from build123d import *


with BuildPart() as part:
    # Sketch1 → Revolve2 (revolve)
    with BuildSketch(Plane.XY, mode=Mode.PRIVATE) as revolve2_sk:
        with BuildLine():
            Line((-2, 0), (-2, 53.291796068))
            ThreePointArc((-2, 53.291796068), (-5.61248608, 55.816699867), (-7, 60))
            Line((-7, 60), (-8, 60))
            Line((-8, 60), (-8, 8.392398037))
            Line((-8, 8.392398037), (-6.75, 8.392398037))
            ThreePointArc((-6.75, 8.392398037), (-6.244894811, 3.375866985), (-2.5, 0))
            Line((-2.5, 0), (-2, 0))
        make_face()
    revolve(revolve2_sk.sketch.rotate(Axis((0, 0, 0), (0, 1, 0)), 270), axis=Axis((0, 0, 0), (0, 1, 0)))


solid = part.part
Could you check a few things on this model? Use its own coordinates, in mm. A direction names the side the tool comes from. Give positions to 0.01 mm unless a question says otherwise; leave off trailing zeros. Loops run counter-clockwise (first coordinate to the right, second up) from the corner with the lowest first, then second, coordinate; pieces in that order, holes last. Notation, with made-up numbers: (50, 11) -> (96, 11) arc R20 ccw to (96, 23) -> close; hole circle Ø7 at (-14, 78.5). An arc over 180 degrees is marked (long way). Return JSON: item names as keys, results as strings.
Item 1: If we section it at D-D on z = -5: List the corners of the cut face in (x, y) for me (3 decimals), plus the area to 3 significant figures.
Geometry results:
{"outline": "(-6.245, 8.392) -> (-4.535, 8.392) arc R4.899 ccw (long way) to (4.535, 8.392) -> (6.245, 8.392) -> (6.245, 60) -> (4.899, 60) arc R4.899 cw to (-4.899, 60) -> (-6.245, 60) -> close", "area": "662 mm²"}
Item 2: If we section it at C-C on y = 19: List the corners of the cut face in (x, z) for me, plus the area to 3 significant figures.
Geometry results:
{"outline": "circle Ø16 at (0, 0); hole circle Ø4 at (0, 0)", "area": "188 mm²"}
Item 3: I'm going to push flat-ended pins straight in: pin 1 (4 mm diameter, centred on y = 50, z = 3, fed in from +X); pin 2 (5 mm diameter, centred on x = 5.5, y = 41.5, fed in from +Z); pin 3 (6 mm diameter, centred on y = 14, z = -5.5, fed in from +X). Where does each tip first touch, or does it pass through?
Geometry results:
{"pin 1": "stops at x = 7.94", "pin 2": "stops at z = 7.42", "pin 3": "stops at x = 7.6"}
Item 4: If we section it at B-B on x = 0: List the corners of the cut face in (y, z) for me, plus the area to 3 significant figures.
Geometry results:
{"outline": "(0, -2.5) arc R7 ccw to (8.39, -6.75) -> (8.39, -8) -> (60, -8) -> (60, -7) arc R7 cw to (53.29, -2) -> (0, -2) -> close; (0, 2) -> (53.29, 2) arc R7 cw to (60, 7) -> (60, 8) -> (8.39, 8) -> (8.39, 6.75) arc R7 ccw to (0, 2.5) -> close", "area": "637 mm²"}
Item 5: We'd pull the mould along Z, two halves only. Please class faces 3 (the cylindrical face through (2, 27, 0)), 4 (the cylindrical face through (7.81, 33.83, 1.73)), 5 (the flat face through (6, 60, 4)): +Z half, -Z half, draft (parallel to the pull), parting line (faces both ways), or undercut.
Geometry results:
{"face 3": "undercut", "face 4": "parting line", "face 5": "draft"}
Item 6: I need wall thicknesses on L1, parallel to X at y = 23, z = 0; L2, parallel to X at y = 44, z = -1.5; L3, parallel to Y at x = 6.75, z = -3.5. Which ranges of each line are inside material? Lowest first, please. Write a range as from..to.
Geometry results:
{"L1": "x = -8..-2, 2..8", "L2": "x = -7.86..-1.32, 1.32..7.86", "L3": "y = 8.39..60"}
Item 7: Which directions (+Z, -Z, +X, -X, +Y, -Y) give clear straight access to the entire face, cutting with the end or side of a thin tool? Please do faces 1 (the flat face through (-2, 0, 1)), 2 (the flat face through (6, 8.392, 4)).
Geometry results:
{"face 1": "+Z, -Z, +X, -X, -Y", "face 2": "none"}
Item 8: If we section it at A-A on z = 0: List the corners of the cut face in (x, y) for me.
Geometry results:
{"outline": "(-8, 8.39) -> (-6.75, 8.39) arc R7 ccw to (-2.5, 0) -> (-2, 0) -> (-2, 53.29) arc R7 cw to (-7, 60) -> (-8, 60) -> close; (2, 0) -> (2.5, 0) arc R7 ccw to (6.75, 8.39) -> (8, 8.39) -> (8, 60) -> (7, 60) arc R7 cw to (2, 53.29) -> close"}
